from build123d import *

# Parameters (mm, degrees)
GB_T6728_2002_70_70_5_1_DEPTH = 1116
CUT_EXTRUDE_1_DEPTH           = 1119.740810018
CUT_EXTRUDE_1_DEPTH_BACK      = 1119.740810018


with BuildPart() as part:
    # Sketch1 → 结构用冷弯空心方钢(gb t6728-2002) 70×70×5(1) (new body)
    with BuildSketch(Plane(origin=(0, 0, 0), x_dir=(-1, 0, 0), z_dir=(0, 1, 0))):
        with BuildLine():
            Line((-25, -35), (25, -35))
            ThreePointArc((25, -35), (32.071067812, -32.071067812), (35, -25))
            Line((35, -25), (35, 25))
            ThreePointArc((35, 25), (32.071067812, 32.071067812), (25, 35))
            Line((25, 35), (-25, 35))
            ThreePointArc((-25, 35), (-32.071067812, 32.071067812), (-35, 25))
            Line((-35, 25), (-35, -25))
            ThreePointArc((-35, -25), (-32.071067812, -32.071067812), (-25, -35))
        make_face()
        with BuildLine():
            Line((-25, -30), (25, -30))
            ThreePointArc((25, -30), (28.535533906, -28.535533906), (30, -25))
            Line((30, -25), (30, 25))
            ThreePointArc((30, 25), (28.535533906, 28.535533906), (25, 30))
            Line((25, 30), (-25, 30))
            ThreePointArc((-25, 30), (-28.535533906, 28.535533906), (-30, 25))
            Line((-30, 25), (-30, -25))
            ThreePointArc((-30, -25), (-28.535533906, -28.535533906), (-25, -30))
        make_face(mode=Mode.SUBTRACT)
    extrude(amount=GB_T6728_2002_70_70_5_1_DEPTH)

    # 草图2 → 切除-拉伸1 (cut, two sides: drawn at the far end of the back side and taken through both)
    with BuildSketch(Plane.XY.offset(35).offset(-CUT_EXTRUDE_1_DEPTH_BACK)):
        Polygon((35, 1116), (-35, 1056.963855422), (-35, 1116), align=None)
        Polygon((-35, 83), (35, 0), (-35, 0), align=None)
    extrude(amount=CUT_EXTRUDE_1_DEPTH + CUT_EXTRUDE_1_DEPTH_BACK, mode=Mode.SUBTRACT)


solid = part.part
Read the model definition and answer for the solid it produces. Units are mm, in the model's axes. A direction names the side the tool comes from. Round coordinates to 2 decimals unless told otherwise and drop trailing zeros. Write each loop counter-clockwise with the first axis right and the second up, starting at its lowest first coordinate (ties: lowest second). Pieces come first, ordered by that corner, then holes.
Q1. Find section B-B on z = 13. Determine the outline of the cut face in (x, y), and give its area (3 significant figures).
Values:
outline: (-35, 83) - (-30, 77.07) - (-30, 1061.18) - (-35, 1056.96) - close; (30, 5.93) - (35, 0) - (35, 1116) - (30, 1111.78) - close
area: 10,400 mm2
Q2. Find section C-C on x = -1. Determine the outline of the cut face in (y, z), and give its area (3 significant figures).
Values:
outline: (42.69, -35) - (1085.64, -35) - (1085.64, -30) - (42.69, -30) - close; (42.69, 30) - (1085.64, 30) - (1085.64, 35) - (42.69, 35) - close
area: 10,400 mm2
Q3. The mould has two halves that part along Z. Classify faces 3 (the face through (-30, 562, 0)), 4 (the face through (0, 552, -35)), 5 (the face through (0, 552, 30)), 6 (the face through (-35, 563, 0)): released by +Z, released by -Z, zero draft, split by the parting line, or undercut.
Values:
face 3: undercut
face 4: released by -Z
face 5: undercut
face 6: zero draft
Q4. A tool of negligible diameter and unlimited length cuts with its end or side. For faces 1 (the face through (0, 552, 35)), 2 (the face through (30, 551, 0)), from which of +Z, -Z, +X, -X, +Y, -Y can it reach the whole face along a straight path? Write none if from no direction.
Values:
face 1: +Z, +X, -X, +Y, -Y
face 2: +Y, -Y
Q5. Straight lines are drawn through the part: line 1 (X direction, y = 937, z = 0); line 2 (X direction, y = 921, z = -27.5). For each, find the intervals that lie inside material, in ascending order.
Values:
line 1: x = -35 to -30, 30 to 35
line 2: x = -34.68 to -29.33, 29.33 to 34.68
Q6. Find section A-A on y = 605. Determine the outline of the cut face in (x, z).
Values:
outline: (-35, -25) arc R10 ccw to (-25, -35) - (25, -35) arc R10 ccw to (35, -25) - (35, 25) arc R10 ccw to (25, 35) - (-25, 35) arc R10 ccw to (-35, 25) - close; hole (-30, -25) arc R5 ccw to (-25, -30) - (25, -30) arc R5 ccw to (30, -25) - (30, 25) arc R5 ccw to (25, 30) - (-25, 30) arc R5 ccw to (-30, 25) - close
